from build123d import *

# Parameters (mm, degrees)
SKETCH_1_W          = 400
SKETCH_1_H          = 365
EXTRUDE_1_DEPTH     = 5
CUT_EXTRUDE_3_DEPTH = 10


with BuildPart() as part:
    # 草图1 → 凸台-拉伸1 (new body)
    with BuildSketch(Plane.XY):
        with Locations((200, 182.5)):
            Rectangle(SKETCH_1_W, SKETCH_1_H)
    extrude(amount=EXTRUDE_1_DEPTH)

    # 草图4 → 切除-拉伸3 (cut)
    with BuildSketch(Plane.XY.offset(5)):
        with BuildLine():
            Line((180, 275), (220, 275))
            ThreePointArc((220, 275), (312.5, 182.5), (220, 90))
            Line((220, 90), (180, 90))
            ThreePointArc((180, 90), (87.5, 182.5), (180, 275))
        make_face()
    extrude(amount=-CUT_EXTRUDE_3_DEPTH, mode=Mode.SUBTRACT)


solid = part.part
Work out the finished part from the listing and answer in its coordinate system (mm). A direction names the side the tool comes from. Round coordinates to 2 decimals unless told otherwise and drop trailing zeros. Loops run counter-clockwise (first coordinate to the right, second up) from the corner with the lowest first, then second, coordinate; pieces in that order, holes last. Notation, with made-up numbers: M 3,22.25 L 28,22.25 A12 cw 28,30.25 Z; hole C -37.5,-37 d2. An arc over 180 degrees is marked long. One line per question, with ' | ' between items. Start each with the question number.
(1) A tool of negligible diameter and unlimited length cuts with its end or side. For faces 3 (the face through (286, 104, 0)), 4 (the face through (87.522, 180.466, 2.535)), from which of +Z, -Z, +X, -X, +Y, -Y can it reach the whole face along a straight path? Write none if from no direction.
(2) A cutting plane is placed at B-B on z = 1.35. Write down the section's boundary in (x, y).
(3) For a pull along X with two mould halves and no side action, classify faces 1 (the face through (312.478, 184.534, 2.535)), 2 (the face through (286, 104, 5)) as released by +X, released by -X, zero draft, split by the parting line, or undercut.
(4) A flat-ended cylindrical pin translates along its axis: pin 1 Ø8 at (x, y) = (230.5, 284) entering from -Z. Find the tip coordinate at first contact, or state that the pin passes through.
(5) Find the intervals of material crossed by line 1 (Y direction, x = 188, z = 0.35); line 2 (X direction, y = 99, z = 1.4); line 3 (X direction, y = 104, z = 0.5), in increasing order.
(6) A cutting plane is placed at A-A on y = 182.5. Write down the section's boundary in (x, z).
(7) A cutting plane is placed at C-C on x = 197. Write down the section's boundary in (y, z), plus the area to 3 significant figures.
Geometry check:
1) face 3: -Z, +X, -X, +Y, -Y | face 4: +Z, -Z
2) outline: M 0,0 L 400,0 L 400,365 L 0,365 Z; hole M 180,90 L 220,90 A92.5 ccw 220,275 L 180,275 A92.5 ccw Z
3) face 1: undercut | face 2: zero draft
4) pin 1: stops at z = 0
5) line 1: y = 0 to 90, 275 to 365 | line 2: x = 0 to 140.2, 259.8 to 400 | line 3: x = 0 to 131.07, 268.93 to 400
6) outline: M 0,0 L 87.5,0 L 87.5,5 L 0,5 Z; M 312.5,0 L 400,0 L 400,5 L 312.5,5 Z
7) outline: M 0,0 L 90,0 L 90,5 L 0,5 Z; M 275,0 L 365,0 L 365,5 L 275,5 Z | area: 900 mm²
